Geometry: final body of the model. Coordinates: model frame, mm. Round coordinates to 2 decimals unless told otherwise and drop trailing zeros. Loops run counter-clockwise (first coordinate to the right, second up) from the corner with the lowest first, then second, coordinate; pieces in that order, holes last. Notation, with made-up numbers: M 46.5,49.5 L 91.5,49.5 A11 ccw 91.5,63.5 Z; hole C -25.5,67 d9. An arc over 180 degrees is marked long. Answer as a JSON object with one key per item and string values.
from build123d import *

# Parameters (mm, degrees)
SKETCH_1_R      = 23.5
SKETCH_1_R_2    = 2.1
EXTRUDE_1_DEPTH = 2


with BuildPart() as part:
    # 草图1 → 凸台-拉伸1 (new body)
    with BuildSketch(Plane(origin=(0, 0, 0), x_dir=(1, 0, 0), z_dir=(0, 1, 0))):
        with BuildLine():
            Line((-31, -13.564659966), (-31, 13.564659966))
            ThreePointArc((-31, 13.564659966), (-30.591663047, 16.393087091), (-29.4, 18.990523953))
            ThreePointArc((-29.4, 18.990523953), (35, 0), (-29.4, -18.990523953))
            ThreePointArc((-29.4, -18.990523953), (-30.591663047, -16.393087091), (-31, -13.564659966))
        make_face()
        with Locations(Location((0, 0, 0), (0, 0, 270))):
            Circle(SKETCH_1_R, mode=Mode.SUBTRACT)
        with Locations(Location((0, 31, 0), (0, 0, 270))):
            Circle(SKETCH_1_R_2, mode=Mode.SUBTRACT)
        with Locations(Location((26.846787517, 15.5, 0), (0, 0, 270))):
            Circle(SKETCH_1_R_2, mode=Mode.SUBTRACT)
        with Locations(Location((26.846787517, -15.5, 0), (0, 0, 270))):
            Circle(SKETCH_1_R_2, mode=Mode.SUBTRACT)
        with Locations(Location((0, -31, 0), (0, 0, 270))):
            Circle(SKETCH_1_R_2, mode=Mode.SUBTRACT)
        with Locations(Location((-26.846787517, -15.5, 0), (0, 0, 270))):
            Circle(SKETCH_1_R_2, mode=Mode.SUBTRACT)
        with Locations(Location((-26.846787517, 15.5, 0), (0, 0, 270))):
            Circle(SKETCH_1_R_2, mode=Mode.SUBTRACT)
    extrude(amount=EXTRUDE_1_DEPTH)


solid = part.part
1) Pin query (flat end, axial travel): P1, Ø5.5, axis at x = 26.85, z = 15.5, coming from the +Y side; P2, Ø4, axis at x = 0, z = 31, coming from the -Y side. Return the tip coordinate at first contact, or that it passes through.
Results:
{"P1": "y = 2", "P2": "through"}
2) Section query D-D (z = -15.5). Return the cut outline in (x, y), and give its area (3 significant figures).
Results:
{"outline": "M -30.81,0 L -28.95,0 L -28.95,2 L -30.81,2 Z; M -24.75,0 L -17.66,0 L -17.66,2 L -24.75,2 Z; M 17.66,0 L 24.75,0 L 24.75,2 L 17.66,2 Z; M 28.95,0 L 31.38,0 L 31.38,2 L 28.95,2 Z", "area": "36.9 mm2"}
3) Section query A-A (x = 0). Return the cut outline in (y, z).
Results:
{"outline": "M 0,-35 L 2,-35 L 2,-33.1 L 0,-33.1 Z; M 0,-28.9 L 2,-28.9 L 2,-23.5 L 0,-23.5 Z; M 0,23.5 L 2,23.5 L 2,28.9 L 0,28.9 Z; M 0,33.1 L 2,33.1 L 2,35 L 0,35 Z"}
4) Section query C-C (x = 20.5). Return the cut outline in (y, z).
Results:
{"outline": "M 0,-28.37 L 2,-28.37 L 2,-11.49 L 0,-11.49 Z; M 0,11.49 L 2,11.49 L 2,28.37 L 0,28.37 Z"}
5) Pull-direction query (Z, two-part tool) for faces 1 (the flat face through (24, 2, 0)), 2 (the cylindrical face through (-24.765, 0.986, 15.227)), 3 (the cylindrical face through (24.797, 0.986, -15.955)), 4 (the cylindrical face through (-30.603, 0.986, -16.355)); classes: +Z half, -Z half, draft (parallel to the pull), parting line (faces both ways), or undercut.
Results:
{"face 1": "draft", "face 2": "undercut", "face 3": "undercut", "face 4": "-Z half"}
6) Ray query, line 1 (X direction, y = 0.85, z = -15.5); line 2 (Z direction, x = -5.5, y = 1.7); line 3 (Z direction, x = -4, y = 1.85). Return the intervals inside material, ascending.
Results:
{"line 1": "-30.81 to -28.95, -24.75 to -17.66, 17.66 to 24.75, 28.95 to 31.38", "line 2": "-34.57 to -22.85, 22.85 to 34.57", "line 3": "-34.77 to -23.16, 23.16 to 34.77"}
7) Section query B-B (z = 0). Return the cut outline in (x, y), and give its area (3 significant figures).
Results:
{"outline": "M -31,0 L -23.5,0 L -23.5,2 L -31,2 Z; M 23.5,0 L 35,0 L 35,2 L 23.5,2 Z", "area": "38.0 mm2"}
